Geometry: final body of the model. Coordinates: model frame, mm. A direction names the side the tool comes from. Coordinates: 2 decimals unless noted, no trailing zeros. Order: outer loops, then holes, each group sorted by start corner. A loop starts at its lowest first (then second) coordinate and runs counter-clockwise, first axis right, second up. Notation, with made-up numbers: M 24,56 L 41,56 A11 ccw 41,62 Z; hole C 88,80 d6. An arc over 180 degrees is marked long. Write item = value, one per line.
from build123d import *

# Parameters (mm, degrees)
BASE_FLANGE_PROFILE_R     = 8
BASE_FLANGE_3MM_DEPTH     = 3
RAISED_PLATE_3MM_DEPTH    = 3
LOBE_CUT_PROFILE_3X_R     = 8
LOBE_CUT_3X_13MM_DEPTH    = 13
BOSSES_3X_DEPTH           = 12
BOSSES_3X_DEPTH_BACK      = 6
BOSS_PROFILE_3X_R         = 8
BOSS_HOLE_PROFILE_3X_R    = 5.5
BOSS_HOLE_PROFILE_3X_R_2  = 3
BOSS_HOLES_3X_12MM_DEPTH  = 12
THROUGH_CUT_PROFILE_3X_R  = 3
THROUGH_CUT_3X_22MM_DEPTH = 22


with BuildPart() as part:
    # Base Flange Profile → Base Flange 3mm (new body)
    with BuildSketch(Plane(origin=(0, 0, 0), x_dir=(1, 0, 0), z_dir=(0, 1, 0))):
        with BuildLine():
            ThreePointArc((14.941453584, 44.323995772), (0, 58), (-14.941453584, 44.323995772))
            ThreePointArc((-14.941453584, 44.323995772), (-16.147655157, 40.973517523), (-18.846153454, 38.65))
            ThreePointArc((-18.846153454, 38.65), (-37.239092363, 21.5), (-42.894958583, -3.003752345))
            ThreePointArc((-42.894958583, -3.003752345), (-43.557934635, -6.502479184), (-45.856433127, -9.222319513))
            ThreePointArc((-45.856433127, -9.222319513), (-50.229473419, -29), (-30.914979544, -35.101676259))
            ThreePointArc((-30.914979544, -35.101676259), (-27.410279478, -34.471038339), (-24.048805129, -35.646247655))
            ThreePointArc((-24.048805129, -35.646247655), (0, -43), (24.048805129, -35.646247655))
            ThreePointArc((24.048805129, -35.646247655), (27.410279478, -34.471038339), (30.914979544, -35.101676259))
            ThreePointArc((30.914979544, -35.101676259), (50.229473419, -29), (45.856433127, -9.222319513))
            ThreePointArc((45.856433127, -9.222319513), (43.557934635, -6.502479184), (42.894958583, -3.003752345))
            ThreePointArc((42.894958583, -3.003752345), (37.239092363, 21.5), (18.846153454, 38.65))
            ThreePointArc((18.846153454, 38.65), (16.147655157, 40.973517523), (14.941453584, 44.323995772))
        make_face()
        with Locations(Location((0, 43, 0), (0, 0, 270))):
            Circle(BASE_FLANGE_PROFILE_R, mode=Mode.SUBTRACT)
        with Locations(Location((37.239092363, -21.5, 0), (0, 0, 270))):
            Circle(BASE_FLANGE_PROFILE_R, mode=Mode.SUBTRACT)
        with Locations(Location((-37.239092363, -21.5, 0), (0, 0, 270))):
            Circle(BASE_FLANGE_PROFILE_R, mode=Mode.SUBTRACT)
    extrude(amount=BASE_FLANGE_3MM_DEPTH)

    # Raised Plate Profile → Raised Plate 3mm (add)
    with BuildSketch(Plane(origin=(0, 3, 0), x_dir=(1, 0, 0), z_dir=(0, 1, 0))):
        with BuildLine():
            ThreePointArc((39.902287054, -2.794188228), (40.8493957, -7.792369426), (44.132964974, -11.67785561))
            ThreePointArc((44.132964974, -11.67785561), (47.631397208, -27.5), (32.179802107, -32.381341007))
            ThreePointArc((32.179802107, -32.381341007), (27.173087728, -31.480429693), (22.370981516, -33.159300144))
            ThreePointArc((22.370981516, -33.159300144), (0, -40), (-22.370981516, -33.159300144))
            ThreePointArc((-22.370981516, -33.159300144), (-27.173087728, -31.480429693), (-32.179802107, -32.381341007))
            ThreePointArc((-32.179802107, -32.381341007), (-47.631397208, -27.5), (-44.132964974, -11.67785561))
            ThreePointArc((-44.132964974, -11.67785561), (-40.8493957, -7.792369426), (-39.902287054, -2.794188228))
            ThreePointArc((-39.902287054, -2.794188228), (-34.641016151, 20), (-17.531305538, 35.953488372))
            ThreePointArc((-17.531305538, 35.953488372), (-13.676307972, 39.272799119), (-11.953162867, 44.059196617))
            ThreePointArc((-11.953162867, 44.059196617), (0, 55), (11.953162867, 44.059196617))
            ThreePointArc((11.953162867, 44.059196617), (13.676307972, 39.272799119), (17.531305538, 35.953488372))
            ThreePointArc((17.531305538, 35.953488372), (34.641016151, 20), (39.902287054, -2.794188228))
        make_face()
    extrude(amount=RAISED_PLATE_3MM_DEPTH)

    # Lobe Cut Profile 3x → Lobe Cut 3x 13mm (cut)
    with BuildSketch(Plane.XZ):
        with Locations(Location((0, -43, 0), (0, 0, 90))):
            Circle(LOBE_CUT_PROFILE_3X_R)
        with Locations(Location((37.239092363, 21.5, 0), (0, 0, 90))):
            Circle(LOBE_CUT_PROFILE_3X_R)
        with Locations(Location((-37.239092363, 21.5, 0), (0, 0, 90))):
            Circle(LOBE_CUT_PROFILE_3X_R)
    extrude(amount=-LOBE_CUT_3X_13MM_DEPTH, mode=Mode.SUBTRACT)

    # Boss Profile 3x → Bosses 3x (add, two sides: drawn at the far end of the back side and taken through both)
    with BuildSketch(Plane(origin=(0, 6, 0), x_dir=(1, 0, 0), z_dir=(0, 1, 0)).offset(-BOSSES_3X_DEPTH_BACK)):
        with Locations(Location((0, 43, 0), (0, 0, 270))):
            Circle(BOSS_PROFILE_3X_R)
        with Locations(Location((37.239092363, -21.5, 0), (0, 0, 270))):
            Circle(BOSS_PROFILE_3X_R)
        with Locations(Location((-37.239092363, -21.5, 0), (0, 0, 270))):
            Circle(BOSS_PROFILE_3X_R)
    extrude(amount=BOSSES_3X_DEPTH + BOSSES_3X_DEPTH_BACK)

    # Boss Hole Profile 3x → Boss Holes 3x 12mm (cut)
    # profile 1 of 3: a face of its own
    with BuildSketch(Plane.XZ):
        with Locations(Location((0, -43, 0), (0, 0, 270))):
            Circle(BOSS_HOLE_PROFILE_3X_R)
        with Locations(Location((0, -43, 0), (0, 0, 270))):
            Circle(BOSS_HOLE_PROFILE_3X_R_2, mode=Mode.SUBTRACT)
    # profile 2 of 3: a face of its own
    with BuildSketch(Plane.XZ):
        with Locations(Location((37.239092363, 21.5, 0), (0, 0, 270))):
            Circle(BOSS_HOLE_PROFILE_3X_R)
        with Locations(Location((37.239092363, 21.5, 0), (0, 0, 270))):
            Circle(BOSS_HOLE_PROFILE_3X_R_2, mode=Mode.SUBTRACT)
    # profile 3 of 3: a face of its own
    with BuildSketch(Plane.XZ):
        with Locations(Location((-37.239092363, 21.5, 0), (0, 0, 270))):
            Circle(BOSS_HOLE_PROFILE_3X_R)
        with Locations(Location((-37.239092363, 21.5, 0), (0, 0, 270))):
            Circle(BOSS_HOLE_PROFILE_3X_R_2, mode=Mode.SUBTRACT)
    extrude(amount=-BOSS_HOLES_3X_12MM_DEPTH, mode=Mode.SUBTRACT)

    # Through Cut Profile 3x → Through Cut 3x 22mm (cut)
    with BuildSketch(Plane.XZ):
        with Locations(Location((0, -43, 0), (0, 0, 270))):
            Circle(THROUGH_CUT_PROFILE_3X_R)
        with Locations(Location((37.239092363, 21.5, 0), (0, 0, 270))):
            Circle(THROUGH_CUT_PROFILE_3X_R)
        with Locations(Location((-37.239092363, 21.5, 0), (0, 0, 270))):
            Circle(THROUGH_CUT_PROFILE_3X_R)
    extrude(amount=-THROUGH_CUT_3X_22MM_DEPTH, mode=Mode.SUBTRACT)


solid = part.part
1) Section C-C, the plane y = 7.75. Return loops of the section in (x, z).
Numbers:
outline = C -37.24,21.5 d16; C 0,-43 d16; C 37.24,21.5 d16; hole C -37.24,21.5 d11; hole C 0,-43 d11; hole C 37.24,21.5 d11
2) Section B-B, the plane z = 21.5. Give the number of separate pieces and of enclosed holes in the cut face, and give its area (3 significant figures).
Numbers:
separate_pieces = 3
enclosed_holes = 0
area = 657 mm²
3) Mould query, pull axis X, two halves, no side actions, for faces 1 (the face through (-35.587, 5.916, 16.254)), 2 (the face through (-4.868, 11.916, -49.349)), 3 (the face through (37.416, 1.479, -21.19)), 4 (the face through (35.41, 14.96, 23.88)). Classes: pulls with the +X half, pulls with the -X half, needs draft (parallel to the pull), parting line crosses it, or undercut.
Numbers:
face_1 = undercut
face_2 = parting line crosses it
face_3 = pulls with the +X half
face_4 = undercut
4) Section D-D, the plane z = -5. Return loops of the section in (x, y).
Numbers:
outline = M -42.71,0 L 42.71,0 L 42.71,3 L 39.69,3 L 39.69,6 L -39.69,6 L -39.69,3 L -42.71,3 Z
5) Set-up query: faces 5 (the face through (0, 4, 40)), 6 (the face through (0, 4, -55)), 7 (the face through (-2.4, 12, -45.4)), 8 (the face through (-13.72, 4.48, -39.21)), 9 (the face through (13.636, 4.479, -39.332)). Return all of +Z, -Z, +X, -X, +Y, -Y with unobstructed straight access to the full face (end or side cutting, diameter ignored); none if empty.
Numbers:
face_5 = +Z, +Y
face_6 = -Z, +Y
face_7 = -Y
face_8 = -Z, -X, +Y
face_9 = -Z, +X, +Y
6) Pin query (flat end, axial travel): pin 1 (5.5 mm diameter, centred on x = 35, z = 23.5, fed in from -Y); pin 2 (1 mm diameter, centred on y = 2.5, z = -26, fed in from +X); pin 3 (8 mm diameter, centred on x = -37.24, z = 21.5, fed in from -Y); pin 4 (5 mm diameter, centred on y = 7, z = 5, fed in from +X). Return the tip coordinate at first contact, or that it passes through.
Numbers:
pin_1 = 0
pin_2 = 34.62
pin_3 = 12
pin_4 = 40.63
7) Section A-A, the plane x = 0. Return loops of the section in (y, z).
Numbers:
outline = M 0,-58 L 3,-58 L 3,-55 L 6,-55 L 6,-51 L 18,-51 L 18,-46 L 12,-46 L 12,-48.5 L 0,-48.5 Z; M 0,-37.5 L 12,-37.5 L 12,-40 L 18,-40 L 18,-35 L 6,-35 L 6,40 L 3,40 L 3,43 L 0,43 Z
8) Line query: L1, parallel to X at y = 9.25, z = 21.5; L2, parallel to X at y = 14, z = 21.5; L3, parallel to Y at x = -5, z = 29.5. Output: solid intervals per line, ascending.
Numbers:
L1 = -45.24 to -42.74, -31.74 to -29.24, 29.24 to 31.74, 42.74 to 45.24
L2 = -45.24 to -40.24, -34.24 to -29.24, 29.24 to 34.24, 40.24 to 45.24
L3 = 0 to 6
